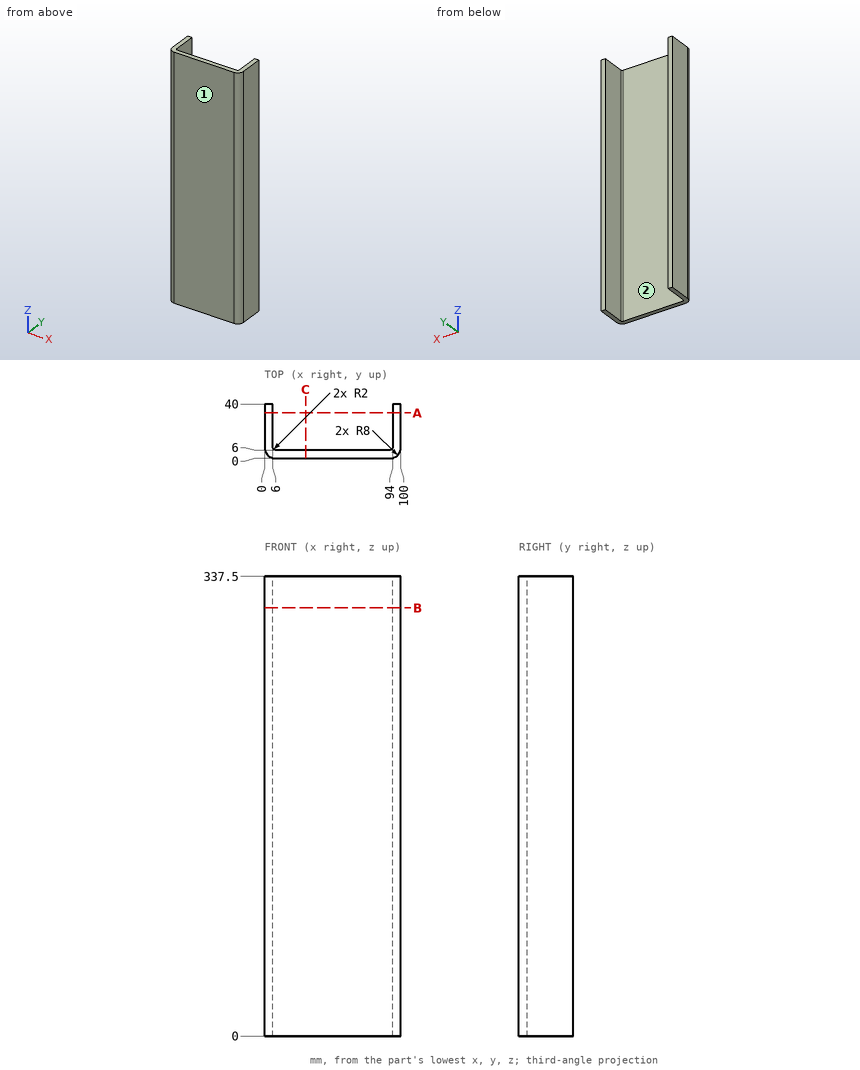
Geometry: see drawing. Coordinates: mm, zero at the bounding-box minimum. A direction names the side the tool comes from. Coordinates: 2 decimals unless noted, no trailing zeros. Loops run counter-clockwise (first coordinate to the right, second up) from the corner with the lowest first, then second, coordinate; pieces in that order, holes last. Notation, with made-up numbers: (84, -37.5) - (98, -37.5) arc R11 cw to (98, -29.5) - close; hole circle Ø5 at (82.5, 56.5). An arc over 180 degrees is marked (long way). Put each result on its own line as item: value. Start each with the question number.
Q1. Set-up query: the marked faces 1 and 2. Return all of +Z, -Z, +X, -X, +Y, -Y with unobstructed straight access to the full face (end or side cutting, diameter ignored); none if empty.
Q2. Cut plane B-B, the plane z = 314.5. Return loops of the section in (x, y).
Q3. Cut plane C-C, the plane x = 30. Return loops of the section in (y, z).
Q4. Pin query (flat end, axial travel): pin 1 Ø5 at (x, z) = (18, 106) entering from +Y. Return the tip coordinate at first contact, or that it passes through.
Q5. Cut plane A-A, the plane y = 33.5. Return loops of the section in (x, z).
Q6. Line query: line 1 (X direction, y = 18, z = 247); line 2 (Y direction, x = 65.5, z = 26); line 3 (X direction, y = 3, z = 301) (3 decimals). Output: solid intervals per line, ascending.
Filled sheet:
1. face 1: +Z, -Z, +X, -X, -Y
1. face 2: +Z, -Z, +Y
2. outline: (0, 8) arc R8 ccw to (8, 0) - (92, 0) arc R8 ccw to (100, 8) - (100, 40) - (94, 40) - (94, 8) arc R2 cw to (92, 6) - (8, 6) arc R2 cw to (6, 8) - (6, 40) - (0, 40) - close
3. outline: (0, 0) - (6, 0) - (6, 337.5) - (0, 337.5) - close
4. pin 1: y = 6
5. outline: (0, 0) - (6, 0) - (6, 337.5) - (0, 337.5) - close; (94, 0) - (100, 0) - (100, 337.5) - (94, 337.5) - close
6. line 1: 0 to 6, 94 to 100
6. line 2: 0 to 6
6. line 3: 1.755 to 98.245
